For this review, take the finished solid that the model builds, in its own axes (mm). Face numbers are marked on the shaded views. A direction names the side the tool comes from. Round coordinates to 2 decimals unless told otherwise and drop trailing zeros. Loops run counter-clockwise (first coordinate to the right, second up) from the corner with the lowest first, then second, coordinate; pieces in that order, holes last. Notation, with made-up numbers: (19, 57.25) -> (70, 57.25) arc R10 ccw to (70, 73.25) -> close; hole circle Ø1 at (43.5, 82). An arc over 180 degrees is marked (long way). Use one line per item in the form item = value. Start each with the question number.
from build123d import *

# Parameters (mm, degrees)
SKETCH_1_W          = 38
SKETCH_1_H          = 38
EXTRUDE_1_DEPTH     = 6
SKETCH_2_R          = 15
EXTRUDE_2_DEPTH     = 3
SKETCH_3_R          = 4
EXTRUDE_3_DEPTH     = 22
SKETCH_4_R          = 19
EXTRUDE_4_DEPTH     = 97
CUT_EXTRUDE_1_REACH = 118.177
SKETCH_5_R          = 1.898690993
CHAMFER_1_SIZE      = 2
CHAMFER_1_SIZE2     = 4


with BuildPart() as part:
    # 草图1 → 拉伸1 (new body)
    with BuildSketch(Plane.XY):
        with Locations((19, 19)):
            Rectangle(SKETCH_1_W, SKETCH_1_H)
    extrude(amount=EXTRUDE_1_DEPTH)

    # 草图2 → 拉伸2 (add)
    with BuildSketch(Plane.XY.offset(6)):
        with Locations(Location((19, 19, 0), (0, 0, 180))):
            Circle(SKETCH_2_R)
    extrude(amount=EXTRUDE_2_DEPTH)

    # 草图3 → 拉伸3 (add)
    with BuildSketch(Plane.XY.offset(9)):
        with Locations((19, 19)):
            Circle(SKETCH_3_R)
    extrude(amount=EXTRUDE_3_DEPTH)

    # 草图4 → 拉伸4 (add)
    with BuildSketch(Plane(origin=(0, 0, 0), x_dir=(-1, 0, 0), z_dir=(0, 0, -1))):
        with Locations((-19, 19)):
            Circle(SKETCH_4_R)
    extrude(amount=EXTRUDE_4_DEPTH)

    # 草图5 → 切除-拉伸1 (cut, up to next)
    with BuildSketch(Plane.XY.offset(6), mode=Mode.PRIVATE) as cut_extrude_1_sk1:
        with Locations((3.090097423, 34.909902577)):
            Circle(SKETCH_5_R)
    cut_extrude_1_tool1 = extrude(cut_extrude_1_sk1.sketch, amount=-CUT_EXTRUDE_1_REACH, mode=Mode.PRIVATE) & part.part
    # 草图5 → 切除-拉伸1 (cut, up to next)
    with BuildSketch(Plane.XY.offset(6), mode=Mode.PRIVATE) as cut_extrude_1_sk2:
        with Locations((34.909902577, 34.909902577)):
            Circle(SKETCH_5_R)
    cut_extrude_1_tool2 = extrude(cut_extrude_1_sk2.sketch, amount=-CUT_EXTRUDE_1_REACH, mode=Mode.PRIVATE) & part.part
    # 草图5 → 切除-拉伸1 (cut, up to next)
    with BuildSketch(Plane.XY.offset(6), mode=Mode.PRIVATE) as cut_extrude_1_sk3:
        with Locations((34.909902577, 3.090097423)):
            Circle(SKETCH_5_R)
    cut_extrude_1_tool3 = extrude(cut_extrude_1_sk3.sketch, amount=-CUT_EXTRUDE_1_REACH, mode=Mode.PRIVATE) & part.part
    # 草图5 → 切除-拉伸1 (cut, up to next)
    with BuildSketch(Plane.XY.offset(6), mode=Mode.PRIVATE) as cut_extrude_1_sk4:
        with Locations((3.090097423, 3.090097423)):
            Circle(SKETCH_5_R)
    cut_extrude_1_tool4 = extrude(cut_extrude_1_sk4.sketch, amount=-CUT_EXTRUDE_1_REACH, mode=Mode.PRIVATE) & part.part
    add(cut_extrude_1_tool1.solids().sort_by_distance((3.090097, 34.909903, 6))[0], mode=Mode.SUBTRACT)
    add(cut_extrude_1_tool2.solids().sort_by_distance((34.909903, 34.909903, 6))[0], mode=Mode.SUBTRACT)
    add(cut_extrude_1_tool3.solids().sort_by_distance((34.909903, 3.090097, 6))[0], mode=Mode.SUBTRACT)
    add(cut_extrude_1_tool4.solids().sort_by_distance((3.090097, 3.090097, 6))[0], mode=Mode.SUBTRACT)

    # 倒角1
    chamfer_1_edges = [part.edges().sort_by_distance(p)[0] for p in [
        (38, 19, -97),
    ]]
    chamfer_1_side = [part.faces().sort_by_distance(p)[0] for p in [
        (38, 19, -48.5),
    ]]
    chamfer(chamfer_1_edges, length=CHAMFER_1_SIZE, length2=CHAMFER_1_SIZE2, reference=chamfer_1_side[0])


solid = part.part
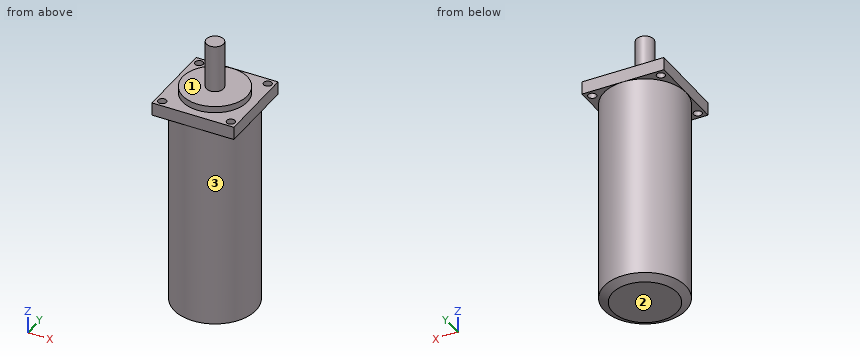
Item 1: Take a section at B-B on z = 13. Give the boundary of the cut face in (x, y).
Item 2: For P1, Ø5, axis at y = 14, z = -58, coming from the -X side; P2, Ø5, axis at x = 31, z = -42, coming from the +Y side; P3, Ø4, axis at x = 11, z = -49.5, coming from the -Y side, all flat-tipped, find the tip position at first contact; note any pin that passes through.
Item 3: Take a section at A-A on z = -84. Give the boundary of the cut face in (x, y).
Item 4: Wall thickness on line 1 (Z direction, x = 24.5, y = 5); line 2 (Z direction, x = 16.5, y = 33); line 3 (Y direction, x = 20.5, z = -24): over which ranges is each line inside the solid? List them lowest first.
Item 5: Machinability: for the marked faces 1, 2 and 3, which of the approach directions +Z, -Z, +X, -X, +Y, -Y give a long, thin tool a straight path to every point of the face, cutting with its end or side? Answer none if there is none.
Results:
q1.outline = circle Ø8 at (19, 19)
q2.P1 = 0.17
q2.P2 = 35.45
q2.P3 = 0.97
q3.outline = circle Ø38 at (19, 19)
q4.line_1 = -96.98 to 6
q4.line_2 = -97 to 9
q4.line_3 = 0.06 to 37.94
q5.face_1 = +Z
q5.face_2 = -Z, +X, -X, +Y, -Y
q5.face_3 = -Z
